Here's the drawing with two shaded views (mm, measured from the low corner). I have some questions. Coordinates: 2 decimals unless noted, no trailing zeros. Loops run counter-clockwise (first coordinate to the right, second up) from the corner with the lowest first, then second, coordinate; pieces in that order, holes last. Notation, with made-up numbers: (28.5, -1.5) -> (48.5, -1.5) arc R19 cw to (48.5, 22.5) -> close; hole circle Ø8 at (16.25, 14). An arc over 180 degrees is marked (long way). Answer as a JSON object with one key per item and string values. Group by question number.
Q1. I want a section at B-B on x = 12.7. Write out the boundary of the cut face in (y, z).
Q2. I want a section at D-D on z = 14. Write out the boundary of the cut face in (x, y).
Q3. I want a section at A-A on z = 7.5. Write out the boundary of the cut face in (x, y).
Q4. I need wall thicknesses on line 1 (Z direction, x = 3, y = 12.7); line 2 (X direction, y = 1.5, z = 10.5); line 3 (X direction, y = 22.75, z = 9). Which ranges of each line are inside material? Lowest first, please.
Q5. Thinking about a two-plate mould opening in X: for the marked faces 1, 2, 3 and 4, which applies, released by +X, released by -X, zero draft, split by the parting line, or undercut?
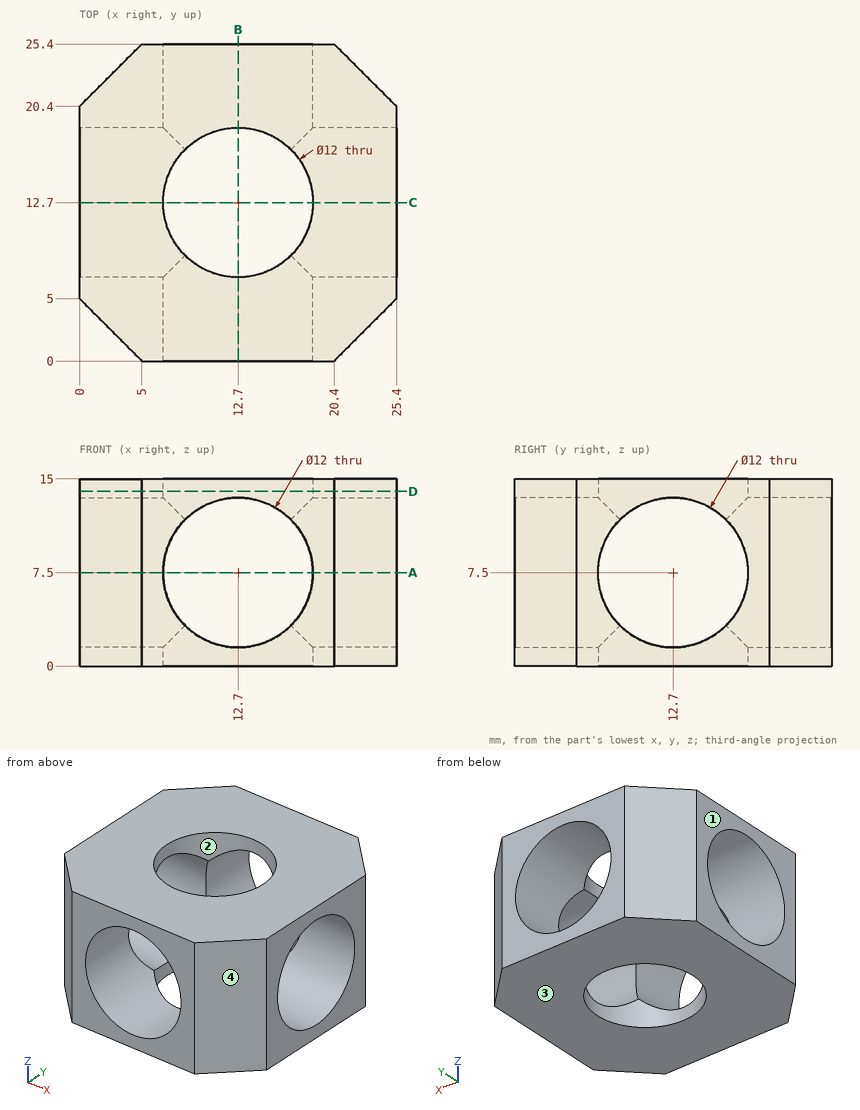
Result set:
{
 "1": {"outline": "(0, 0) -> (6.7, 0) -> (6.7, 1.5) -> (0, 1.5) -> close; (0, 13.5) -> (6.7, 13.5) -> (6.7, 15) -> (0, 15) -> close; (18.7, 0) -> (25.4, 0) -> (25.4, 1.5) -> (18.7, 1.5) -> close; (18.7, 13.5) -> (25.4, 13.5) -> (25.4, 15) -> (18.7, 15) -> close"},
 "2": {"outline": "(0, 5) -> (5, 0) -> (20.4, 0) -> (25.4, 5) -> (25.4, 20.4) -> (20.4, 25.4) -> (5, 25.4) -> (0, 20.4) -> close; hole circle Ø12 at (12.7, 12.7)"},
 "3": {"outline": "(0, 5) -> (5, 0) -> (6.7, 0) -> (6.7, 6.7) -> (0, 6.7) -> close; (0, 18.7) -> (6.7, 18.7) -> (6.7, 25.4) -> (5, 25.4) -> (0, 20.4) -> close; (18.7, 0) -> (20.4, 0) -> (25.4, 5) -> (25.4, 6.7) -> (18.7, 6.7) -> close; (18.7, 18.7) -> (25.4, 18.7) -> (25.4, 20.4) -> (20.4, 25.4) -> (18.7, 25.4) -> close"},
 "4": {"line 1": "z = 0 to 1.5, 13.5 to 15", "line 2": "x = 3.5 to 7.5, 17.9 to 21.9", "line 3": "x = 2.35 to 6.89, 18.51 to 23.05"},
 "5": {"face 1": "released by -X", "face 2": "undercut", "face 3": "zero draft", "face 4": "released by +X"}
}
